Part print with two shaded views. Sizes in mm from the minimum x, y, z corner. A direction names the side the tool comes from. Round coordinates to 2 decimals unless told otherwise and drop trailing zeros. Loops run counter-clockwise (first coordinate to the right, second up) from the corner with the lowest first, then second, coordinate; pieces in that order, holes last.
(1) Cut at C-C on z = 27. List the corners of the cut face in (x, y), then the cut area to 3 significant figures.
(2) Cut at A-A on x = 30. List the corners of the cut face in (y, z), then the cut area to 3 significant figures.
(3) Mould opens along Z. For the marked faces 1, 2, 3 and 4 say: +Z half, -Z half, draft (parallel to the pull), parting line (faces both ways), or undercut.
(4) Flat gauge pins, fed straight in: pin 1 (2 mm diameter, centred on x = 49.5, z = 24, fed in from +Y); pin 2 (5 mm diameter, centred on x = 10.5, y = 9.5, fed in from +Z). Where does each tip first touch, or does it go through?
(5) Cut at D-D on x = 22. List the corners of the cut face in (y, z).
(6) Tool access for the marked faces 5 and 6: list every direction of +Z, -Z, +X, -X, +Y, -Y with a clear straight run to the whole face (end or side of a thin tool).
(7) Cut at B-B on y = 30. Count the separate pieces of the cut face and the enclosed holes in it, then the cut area to 3 significant figures.
(8) Probe probe 1 along Y at (x, z) = (30, 1); probe 2 along Z at (x, y) = (27, 20.5); probe 3 along Z at (x, y) = (52, 30.5). List the from-to ranges inside material, lowest first.
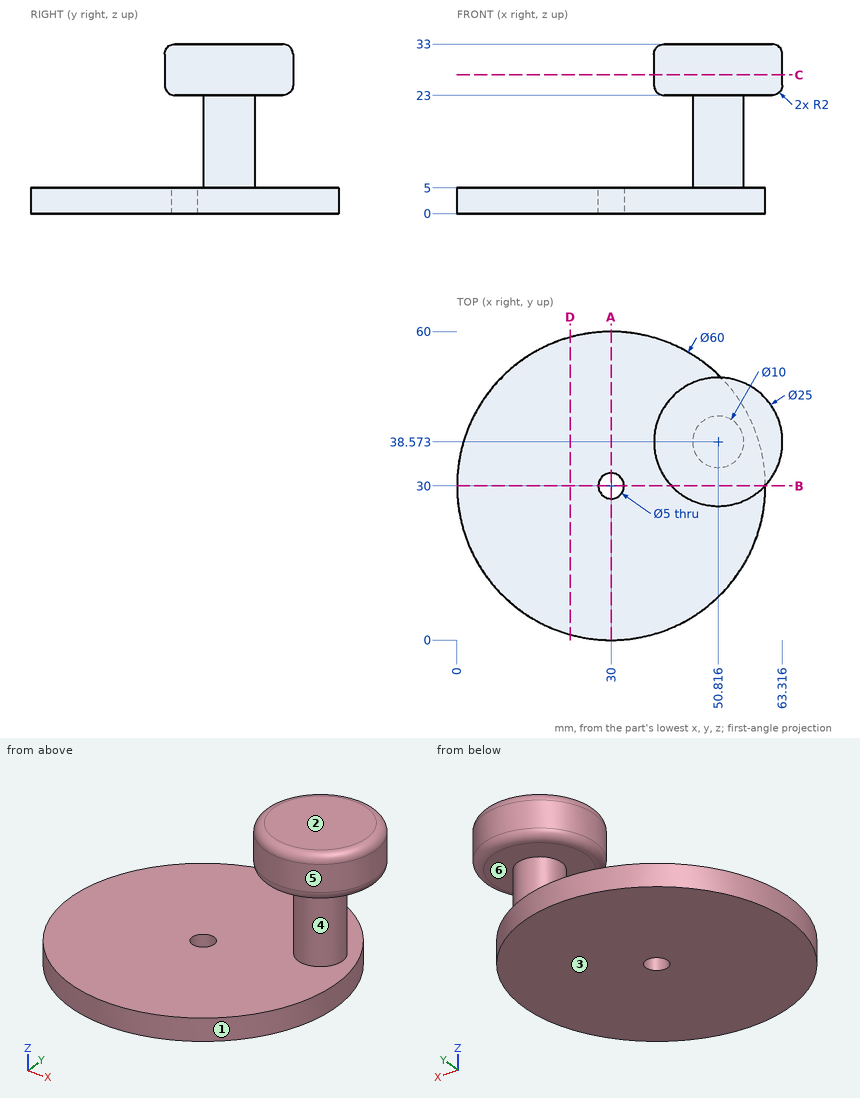
Final values:
1. outline: circle Ø25 at (50.82, 38.57)
1. area: 491 mm2
2. outline: (0, 0) - (27.5, 0) - (27.5, 5) - (0, 5) - close; (32.5, 0) - (60, 0) - (60, 5) - (32.5, 5) - close
2. area: 275 mm2
3. face 1: draft
3. face 2: +Z half
3. face 3: -Z half
3. face 4: undercut
4. pin 1: stops at y = 51.04
4. pin 2: stops at z = 5
5. outline: (1.09, 0) - (58.91, 0) - (58.91, 5) - (1.09, 5) - close
6. face 5: +Z
6. face 6: none
7. separate pieces: 3
7. enclosed holes: 0
7. area: 452 mm2
8. probe 1: y = 0 to 27.5, 32.5 to 60
8. probe 2: z = 0 to 5
8. probe 3: z = 0 to 5, 23 to 33
